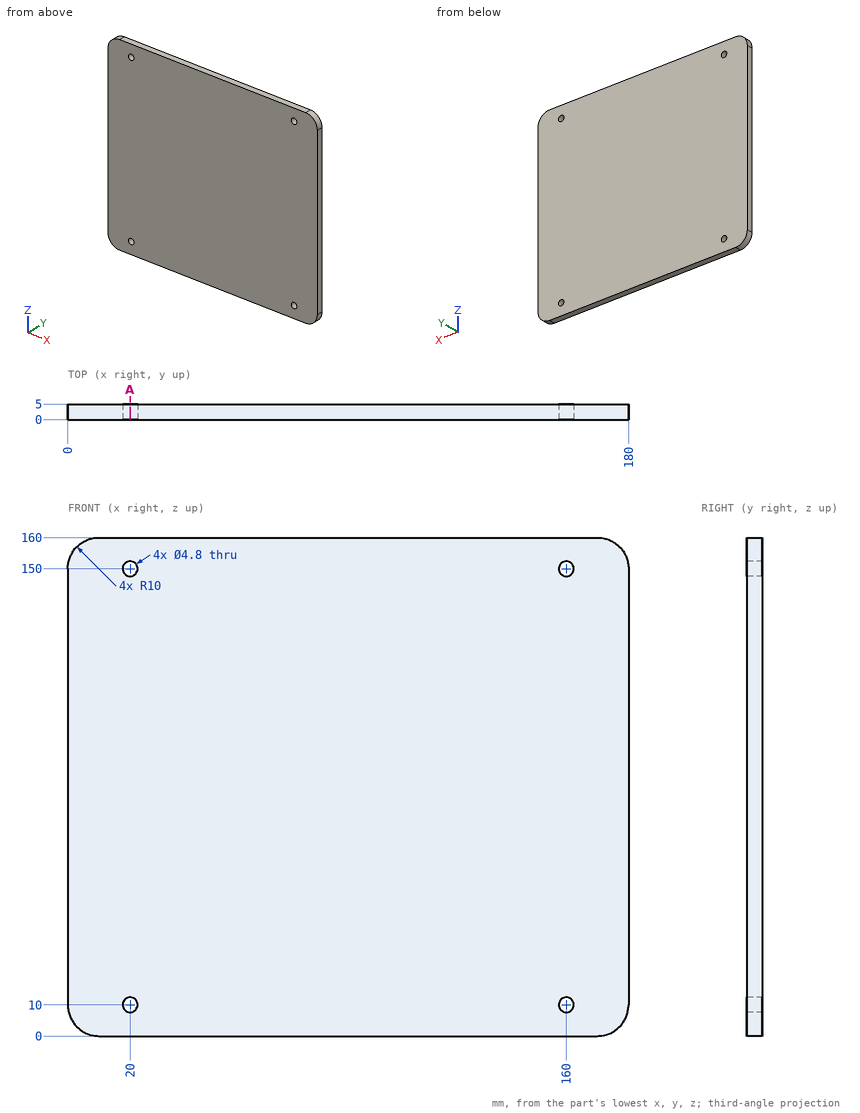
Can you work these out from the drawing? Everything is in mm from the part's minimum corner. Give positions to 0.01 mm unless a question says otherwise; leave off trailing zeros. Order: outer loops, then holes, each group sorted by start corner. A loop starts at its lowest first (then second) coordinate and runs counter-clockwise, first axis right, second up. Notation, with made-up numbers: M 8,-11.5 L 22,-11.5 A24 ccw 22,10.5 Z; hole C -21,-0.75 d11. An arc over 180 degrees is marked long. One line per item, written item: value.
Item 1: Please list where these lines run through material, in increasing order: line 1 (X direction, y = 1.25, z = 10); line 2 (Z direction, x = 160, y = 1.9).
Verdict:
line 1: 0 to 17.6, 22.4 to 157.6, 162.4 to 180
line 2: 0 to 7.6, 12.4 to 147.6, 152.4 to 160
Item 2: For pin 1 (7.5 mm diameter, centred on x = 160, z = 150, fed in from -Y), with a flat end and sliding along its axis, tell me the tip position at first contact or that it passes through.
Verdict:
pin 1: y = 0
Item 3: If we section it at A-A on x = 20: Write out the boundary of the cut face in (y, z), and give its area (3 significant figures).
Verdict:
outline: M 0,0 L 5,0 L 5,7.6 L 0,7.6 Z; M 0,12.4 L 5,12.4 L 5,147.6 L 0,147.6 Z; M 0,152.4 L 5,152.4 L 5,160 L 0,160 Z
area: 752 mm2
